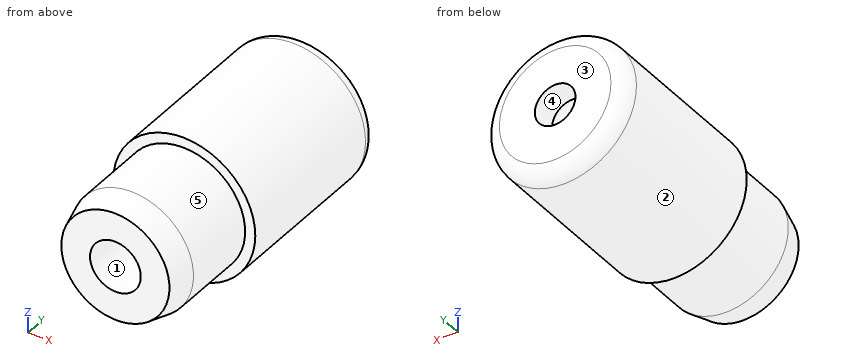
from build123d import *


with BuildPart() as part:
    # Pin Revolve Profile → Pin Body Revolve (revolve)
    with BuildSketch(Plane.XY):
        with BuildLine():
            Line((-4, 60.189864048), (-4, 65.189864048))
            Line((-4, 65.189864048), (-11, 65.189864048))
            ThreePointArc((-11, 65.189864048), (-13.121320344, 64.311184392), (-14, 62.189864048))
            Line((-14, 62.189864048), (-14, 30.189864048))
            Line((-14, 30.189864048), (-12, 30.189864048))
            Line((-12, 30.189864048), (-12, 15.189864048))
            Line((-12, 15.189864048), (-10.660254038, 10.189864048))
            Line((-10.660254038, 10.189864048), (-5, 10.189864048))
            Line((-5, 10.189864048), (-5, 37.189864048))
            Line((-5, 37.189864048), (-4, 38.189864048))
            Line((-4, 38.189864048), (-4, 47.189864048))
            ThreePointArc((-4, 47.189864048), (-5.5, 48.689864048), (-4, 50.189864048))
            Line((-4, 50.189864048), (-4, 57.189864048))
            ThreePointArc((-4, 57.189864048), (-5.5, 58.689864048), (-4, 60.189864048))
        make_face()
    revolve(axis=Axis((0, 148.451497923, 0), (0, -1, 0)))


solid = part.part
The listing builds one solid part. Answer for the finished solid, in the listing's coordinates (mm). Face numbers are marked on the shaded views. A direction names the side the tool comes from. Coordinates: 2 decimals unless noted, no trailing zeros. Order: outer loops, then holes, each group sorted by start corner. A loop starts at its lowest first (then second) coordinate and runs counter-clockwise, first axis right, second up. Notation, with made-up numbers: (-21, 81) -> (38, 81) arc R21 cw to (38, 92) -> close; hole circle Ø1 at (41.5, 66). An arc over 180 degrees is marked (long way). Answer in a Markdown table with one row per item. Add a question column.
Item 1: Which of the six approach directions +Z, -Z, +X, -X, +Y, -Y give full straight-line access (tool end or side, diameter ignored) to the marked faces 4 and 5?
Item 2: Find the intervals of material crossed by L1, parallel to X at y = 40.5, z = 0; L2, parallel to X at y = 22, z = 0, in increasing order. Write a range as from..to.
Item 3: Determine the mould class of the marked faces 1, 2 and 3 for opening direction X: +X half, -X half, draft (parallel to the pull), parting line (faces both ways), or undercut.
Item 4: Find section C-C (y = 25). Write down the section's boundary in (x, z), then the cut area to 3 significant figures.
Item 5: Find section D-D (y = 54). Write down the section's boundary in (x, z).
Item 6: Find section B-B (z = 0). Write down the section's boundary in (x, y).
Item 7: Find section A-A (x = 0). Write down the section's boundary in (y, z), then the cut area to 3 significant figures.
Item 8: Each of these flat-tipped pins is pushed along its axis until it touches: P1, Ø5, axis at y = 16.5, z = 3, coming from the +X side; P2, Ø2, axis at y = 38.5, z = 6.5, coming from the +X side; P3, Ø3, axis at y = 34, z = 5.5, coming from the +X side. Where does it stop, or does it pass through?
Result set:
| question | item | result |
|---|---|---|
| 1 | face 4 | +Y, -Y |
| 1 | face 5 | -Y |
| 2 | L1 | x = -14..-4, 4..14 |
| 2 | L2 | x = -12..-5, 5..12 |
| 3 | face 1 | undercut |
| 3 | face 2 | parting line |
| 3 | face 3 | draft |
| 4 | outline | circle Ø24 at (0, 0); hole circle Ø10 at (0, 0) |
| 4 | area | 374 mm² |
| 5 | outline | circle Ø28 at (0, 0); hole circle Ø8 at (0, 0) |
| 6 | outline | (-14, 30.19) -> (-12, 30.19) -> (-12, 15.19) -> (-10.66, 10.19) -> (-5, 10.19) -> (-5, 37.19) -> (-4, 38.19) -> (-4, 47.19) arc R1.5 cw to (-4, 50.19) -> (-4, 57.19) arc R1.5 cw to (-4, 60.19) -> (-4, 65.19) -> (-11, 65.19) arc R3 ccw to (-14, 62.19) -> close; (4, 38.19) -> (5, 37.19) -> (5, 10.19) -> (10.66, 10.19) -> (12, 15.19) -> (12, 30.19) -> (14, 30.19) -> (14, 62.19) arc R3 ccw to (11, 65.19) -> (4, 65.19) -> (4, 60.19) arc R1.5 cw to (4, 57.19) -> (4, 50.19) arc R1.5 cw to (4, 47.19) -> close |
| 7 | outline | (10.19, -10.66) -> (15.19, -12) -> (30.19, -12) -> (30.19, -14) -> (62.19, -14) arc R3 ccw to (65.19, -11) -> (65.19, -4) -> (60.19, -4) arc R1.5 cw to (57.19, -4) -> (50.19, -4) arc R1.5 cw to (47.19, -4) -> (38.19, -4) -> (37.19, -5) -> (10.19, -5) -> close; (10.19, 5) -> (37.19, 5) -> (38.19, 4) -> (47.19, 4) arc R1.5 cw to (50.19, 4) -> (57.19, 4) arc R1.5 cw to (60.19, 4) -> (65.19, 4) -> (65.19, 11) arc R3 ccw to (62.19, 14) -> (30.19, 14) -> (30.19, 12) -> (15.19, 12) -> (10.19, 10.66) -> close |
| 7 | area | 940 mm² |
| 8 | P1 | stops at x = 11.99 |
| 8 | P2 | stops at x = 12.87 |
| 8 | P3 | stops at x = 13.42 |
